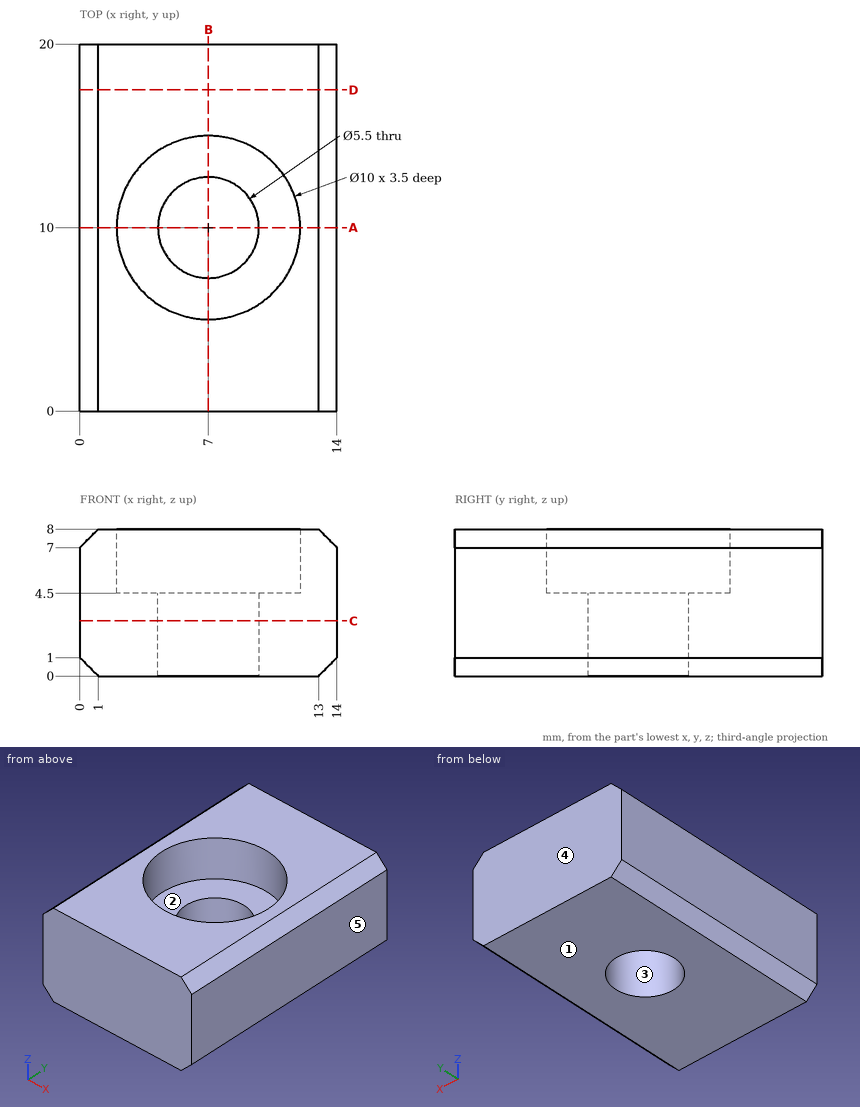
Job drawing, mm, ordinate dimensions from the low corner. One solid piece. A direction names the side the tool comes from. Give positions to 0.01 mm unless a question says otherwise; leave off trailing zeros. Order: outer loops, then holes, each group sorted by start corner. A loop starts at its lowest first (then second) coordinate and runs counter-clockwise, first axis right, second up. Notation, with made-up numbers: (87.5, 21.5) - (146.5, 21.5) arc R20 ccw to (146.5, 55.5) - close; hole circle Ø8 at (-25, -24.75). An arc over 180 degrees is marked (long way). Return JSON: item names as keys, results as strings.
1) Probe line 1 (Y direction, x = 7, z = 3.4); line 2 (Z direction, x = 4, y = 9); line 3 (Y direction, x = 10.5, z = 5.5). List the from-to ranges inside material, lowest first. Write a range as from..to.
Geometry says:
{"line 1": "0..7.25, 12.75..20", "line 2": "0..4.5", "line 3": "0..6.43, 13.57..20"}
2) 3-axis set-ups, long thin cutter, end or side, ignore diameter. For the marked faces 1 and 2: which of +Z, -Z, +X, -X, +Y, -Y reach the whole face in a straight line?
Geometry says:
{"face 1": "-Z, +X, -X, +Y, -Y", "face 2": "+Z"}
3) Cut at D-D, the plane y = 17.5. Give the cut face in (x, z), plus the area to 3 significant figures.
Geometry says:
{"outline": "(0, 1) - (1, 0) - (13, 0) - (14, 1) - (14, 7) - (13, 8) - (1, 8) - (0, 7) - close", "area": "110 mm²"}
4) Pull direction X, two halves, no side cores. Call the marked faces 3, 4 and 5: pulls with the +X half, pulls with the -X half, needs draft (parallel to the pull), parting line crosses it, or undercut.
Geometry says:
{"face 3": "undercut", "face 4": "needs draft", "face 5": "pulls with the +X half"}
5) Cut at B-B, the plane x = 7. Give the cut face in (y, z), plus the area to 3 significant figures.
Geometry says:
{"outline": "(0, 0) - (7.25, 0) - (7.25, 4.5) - (5, 4.5) - (5, 8) - (0, 8) - close; (12.75, 0) - (20, 0) - (20, 8) - (15, 8) - (15, 4.5) - (12.75, 4.5) - close", "area": "100 mm²"}
6) Cut at A-A, the plane y = 10. Give the cut face in (x, z), plus the area to 4 significant figures.
Geometry says:
{"outline": "(0, 1) - (1, 0) - (4.25, 0) - (4.25, 4.5) - (2, 4.5) - (2, 8) - (1, 8) - (0, 7) - close; (9.75, 0) - (13, 0) - (14, 1) - (14, 7) - (13, 8) - (12, 8) - (12, 4.5) - (9.75, 4.5) - close", "area": "50.25 mm²"}
7) Flat gauge pin, fed straight in: P1, Ø5, axis at x = 8.5, y = 10, coming from the +Z side. Where does the tip first touch, or does it go through?
Geometry says:
{"P1": "z = 4.5"}
8) Cut at C-C, the plane z = 3. Give the cut face in (x, y), plus the area to 3 significant figures.
Geometry says:
{"outline": "(0, 0) - (14, 0) - (14, 20) - (0, 20) - close; hole circle Ø5.5 at (7, 10)", "area": "256 mm²"}
